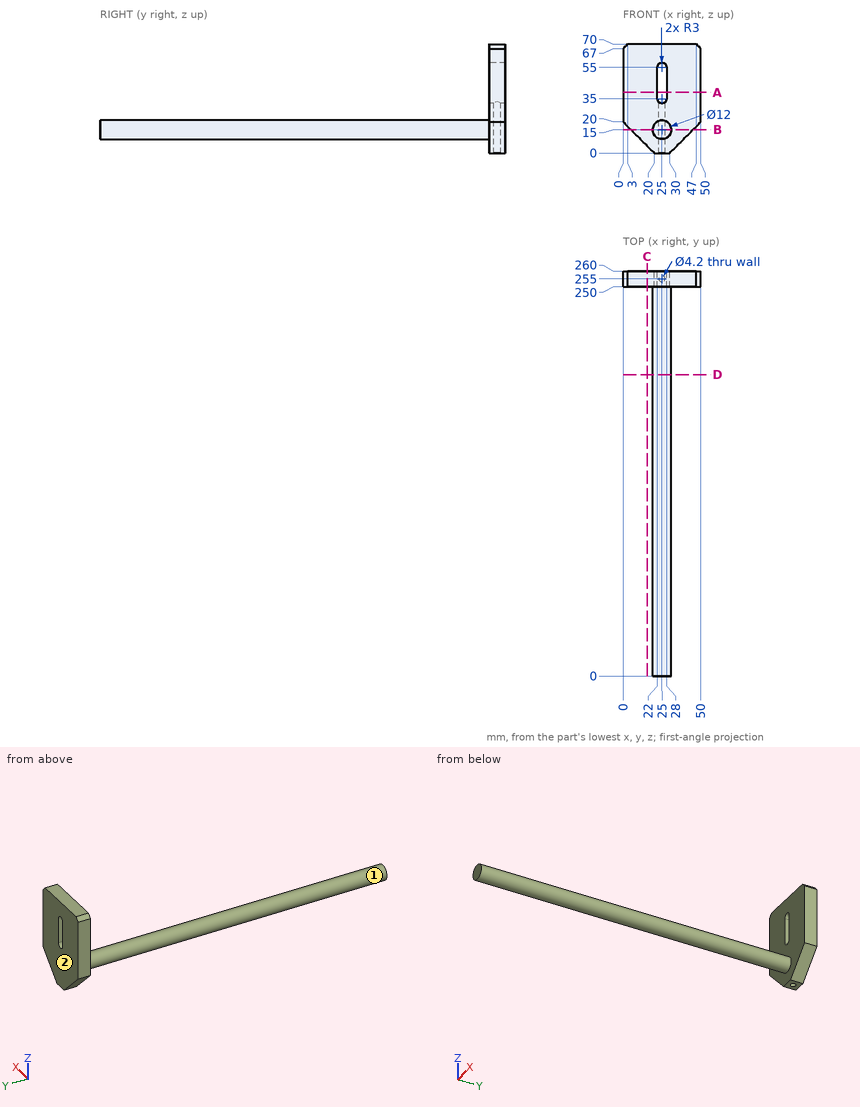
Verification items for this drawing (mm, ordinates from the low corner). A direction names the side the tool comes from. Give positions to 0.01 mm unless a question says otherwise; leave off trailing zeros. Write each loop counter-clockwise with the first axis right and the second up, starting at its lowest first coordinate (ties: lowest second). Pieces come first, ordered by that corner, then holes. Notation, with made-up numbers: (44.5, -25.75) -> (103.5, -25.75) arc R18 cw to (103.5, 4.25) -> close; hole circle Ø8 at (-9.75, 14). An arc over 180 degrees is marked (long way). Use CSV: the item, a comma, the result in double quotes. Start each with the question number.
Q1. Cross-section at D-D on y = 193.5. Enter the section's corners in (x, z), and give its area (3 significant figures).
Q2. Depth check by flat-ended pin: P1, Ø25, axis at x = 17.5, z = 52, coming from the -Y side; P2, Ø1, axis at y = 210, z = 16.5, coming from the +X side; P3, Ø3, axis at y = 170, z = 9.5, coming from the +X side. Enter the tip coordinate at first touch or a pass-through.
Q3. Scan lines: line 1 along X through (y, z) = (255, 23.5); line 2 along Y through (x, z) = (25, 12); line 3 along Y through (x, z) = (32, 8.5). Record each from-to range of solid material in increasing order.
Q4. Tool access check on the marked faces 1 and 2. Record the directions out of +Z, -Z, +X, -X, +Y, -Y that give a thin tool (end or side, any length) a straight path to the whole face; none if there is none.
Q5. Cross-section at B-B on z = 15. Enter the section's corners in (x, y), and give its area (3 significant figures).
Q6. Cross-section at A-A on z = 39. Enter the section's corners in (x, y), and give its area (3 significant figures).
Q7. Cross-section at C-C on x = 15.5. Enter the section's corners in (y, z).
Working result:
1,outline,"circle Ø12 at (25, 15)"
1,area,"113 mm^2"
2,P1,"stops at y = 250"
2,P2,"stops at x = 30.92"
2,P3,"stops at x = 29.47"
3,line 1,"x = 0 to 22.9, 27.1 to 50"
3,line 2,"y = 0 to 252.9, 257.1 to 260"
3,line 3,"y = 250 to 260"
4,face 1,"-Y"
4,face 2,"+Z, -Z, +X, -X, +Y"
5,outline,"(5, 250) -> (19, 250) -> (19, 0) -> (31, 0) -> (31, 250) -> (45, 250) -> (45, 260) -> (5, 260) -> close; hole circle Ø4.2 at (25, 255)"
5,area,"3,390 mm^2"
6,outline,"(0, 250) -> (22, 250) -> (22, 260) -> (0, 260) -> close; (28, 250) -> (50, 250) -> (50, 260) -> (28, 260) -> close"
6,area,"440 mm^2"
7,outline,"(250, 4.5) -> (260, 4.5) -> (260, 70) -> (250, 70) -> close"
